The model under review builds one solid part; all positions refer to its coordinate system, in mm. Face numbers are marked on the shaded views. A direction names the side the tool comes from. Round coordinates to 2 decimals unless told otherwise and drop trailing zeros. Order: outer loops, then holes, each group sorted by start corner. A loop starts at its lowest first (then second) coordinate and runs counter-clockwise, first axis right, second up.
1) Clearance check with flat-ended pins moving along their axes: P1, Ø7.5, axis at x = -1, y = 19.5, coming from the +Z side; P2, Ø3, axis at y = 19.5, z = 0, coming from the -X side; P3, Ø14.5, axis at x = 29, y = 23.5, coming from the -Z side. State where each tip first meets the part, or that it passes through.
2) Consider section C-C (x = 5). Give the boundary of the cut face in (y, z) (3 decimals), then the cut area to 3 significant figures.
3) Mouldability with a two-part tool opening along Y and no side actions: class the marked faces 1, 2 and 3 as pulls with the +Y half, pulls with the -Y half, needs draft (parallel to the pull), parting line crosses it, or undercut.
4) Consider section B-B (y = 4). Give the boundary of the cut face in (x, z), then the cut area to 3 significant figures.
5) Consider section A-A (z = 17). Give the boundary of the cut face in (x, y).
6) To check wall thickness, follow L1, parallel to Y at x = 27, z = 17.25; L2, parallel to Y at x = 0, z = -14; L3, parallel to Y at x = 0, z = -12. State the ranges of each line that lie inside material, in increasing order.
7) Machinability: for the marked faces 4, 5, 6, 7 and 8, which of the approach directions +Z, -Z, +X, -X, +Y, -Y give a long, thin tool a straight path to every point of the face, cutting with its end or side? Answer none if there is none.
8) Consider section D-D (z = -4). Give the boundary of the cut face in (x, y).
from build123d import *

# Parameters (mm, degrees)
BOSS_EXTRUDE1_DEPTH   = 36
FILLET1_R             = 5
FILLET2_R             = 2
SKETCH2_R             = 3.5
CUT_EXTRUDE1_DEPTH    = 59.489315264
SKETCH3_R             = 10
CUT_EXTRUDE2_DEPTH    = 6
SKETCH4_R             = 8
BOSS_EXTRUDE2_DEPTH   = 11.09
M8_TAPPED_HOLE1_D     = 6.8
M8_TAPPED_HOLE1_DEPTH = 22.25
M8_TAPPED_HOLE1_TIP   = 2.042926105
FILLET3_R             = 2


with BuildPart() as part:
    # Sketch1 → Boss-Extrude1 (new body)
    with BuildSketch(Plane(origin=(0, 0, 0), x_dir=(1, 0, 0), z_dir=(0, 1, 0))):
        Polygon((-20, -13.744612069), (-20, 16.255387931), (20, 16.255387931), (20, -13.744612069), (35, -13.744612069), (35, -19.744612069), (18.390996312, -19.744612069), (10, -9.744612069), (-10, -9.744612069), (-18.390996312, -19.744612069), (-35, -19.744612069), (-35, -13.744612069), align=None)
        with BuildLine():
            Line((-10, 13.167446825), (10, 13.167446825))
            ThreePointArc((10, 13.167446825), (12, 11.167446825), (10, 9.167446825))
            Line((10, 9.167446825), (-10, 9.167446825))
            ThreePointArc((-10, 9.167446825), (-12, 11.167446825), (-10, 13.167446825))
        make_face(mode=Mode.SUBTRACT)
    extrude(amount=BOSS_EXTRUDE1_DEPTH)

    # Fillet1
    fillet1_edges = [part.edges().sort_by_distance(p)[0] for p in [
        (18.390996312, 18, 19.744612069),
        (10, 18, 9.744612069),
        (-10, 18, 9.744612069),
        (-18.390996312, 18, 19.744612069),
    ]]
    fillet(fillet1_edges, radius=FILLET1_R)

    # Fillet2
    fillet2_edges = [part.edges().sort_by_distance(p)[0] for p in [
        (20, 18, 13.744612069),
        (-20, 18, 13.744612069),
    ]]
    fillet(fillet2_edges, radius=FILLET2_R)

    # Sketch2 → Cut-Extrude1 (cut, through all)
    with BuildSketch(Plane(origin=(0, 0, 13.744612069), x_dir=(-1, 0, 0), z_dir=(0, 0, -1))):
        with Locations((-27, 18)):
            Circle(SKETCH2_R)
        with Locations((27, 18)):
            Circle(SKETCH2_R)
    extrude(amount=-CUT_EXTRUDE1_DEPTH, mode=Mode.SUBTRACT)

    # Sketch3 → Cut-Extrude2 (cut)
    with BuildSketch(Plane(origin=(0, 0, -16.255387931), x_dir=(-1, 0, 0), z_dir=(0, 0, -1))):
        with Locations((0, 18)):
            Circle(SKETCH3_R)
    extrude(amount=-CUT_EXTRUDE2_DEPTH, mode=Mode.SUBTRACT)

    # Sketch4 → Boss-Extrude2 (add)
    with BuildSketch(Plane(origin=(0, 0, -9.167446825), x_dir=(-1, 0, 0), z_dir=(0, 0, -1))):
        with Locations((0, 18)):
            Circle(SKETCH4_R)
    extrude(amount=BOSS_EXTRUDE2_DEPTH)

    # M8 Tapped Hole1
    with Locations(Plane(origin=(0, 0, -20.257446825), x_dir=(-1, 0, 0), z_dir=(0, 0, -1))):
        with Locations((0, 18)):
            Hole(M8_TAPPED_HOLE1_D / 2, depth=M8_TAPPED_HOLE1_DEPTH)
            with Locations((0, 0, -(M8_TAPPED_HOLE1_DEPTH + M8_TAPPED_HOLE1_TIP / 2))):  # 118° drill point
                Cone(0, M8_TAPPED_HOLE1_D / 2, M8_TAPPED_HOLE1_TIP, mode=Mode.SUBTRACT)

    # Fillet3
    fillet3_edges = [part.edges().sort_by_distance(p)[0] for p in [
        (-20, 18, -16.255387931),
        (20, 18, -16.255387931),
    ]]
    fillet(fillet3_edges, radius=FILLET3_R)


solid = part.part
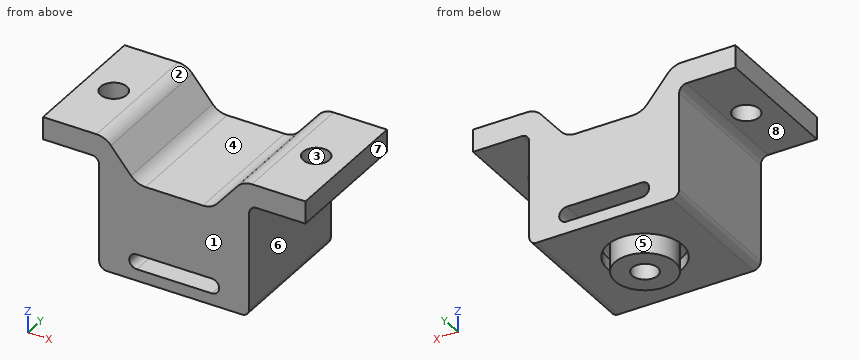
Answer below:
1. P1: stops at z = 9.74
1. P2: stops at x = -20
1. P3: stops at z = 13.73
2. outline: (0, -16.255) - (9.34, -16.255) - (9.34, -13.167) - (0, -13.167) - close; (0, -9.167) - (11.755, -9.167) - (11.755, -20.257) - (24.245, -20.257) - (24.245, -9.167) - (36, -9.167) - (36, 9.745) - (0, 9.745) - close; (26.66, -16.255) - (36, -16.255) - (36, -13.167) - (26.66, -13.167) - close
2. area: 877 mm2
3. face 1: pulls with the -Y half
3. face 2: needs draft
3. face 3: undercut
4. outline: (-35, 13.74) - (-22, 13.74) arc R2 cw to (-20, 11.74) - (-20, -14.26) arc R2 ccw to (-18, -16.26) - (18, -16.26) arc R2 ccw to (20, -14.26) - (20, 11.74) arc R2 cw to (22, 13.74) - (35, 13.74) - (35, 19.74) - (20.72, 19.74) arc R5 ccw to (16.89, 17.96) - (11.5, 11.53) arc R5 cw to (7.67, 9.74) - (-7.67, 9.74) arc R5 cw to (-11.5, 11.53) - (-16.89, 17.96) arc R5 ccw to (-20.72, 19.74) - (-35, 19.74) - close; hole (-10, -13.17) - (10, -13.17) arc R2 ccw to (10, -9.17) - (-10, -9.17) arc R2 ccw to start
4. area: 1,240 mm2
5. outline: (-35, 0) - (-16.09, 0) - (-16.09, 36) - (-35, 36) - close; (16.09, 0) - (35, 0) - (35, 36) - (16.09, 36) - close; hole circle Ø7 at (-27, 18); hole circle Ø7 at (27, 18)
6. L1: y = 0 to 14.5, 21.5 to 36
6. L2: y = 0 to 8, 10 to 14.6, 21.4 to 26, 28 to 36
6. L3: y = 10 to 14.6, 21.4 to 26
7. face 4: +Z, +Y, -Y
7. face 5: -Z
7. face 6: -Z, +X, +Y, -Y
7. face 7: +Z, -Z, +X, +Y, -Y
7. face 8: -Z, -X, +Y, -Y
8. outline: (-20, 0) - (20, 0) - (20, 36) - (-20, 36) - close; hole circle Ø6.8 at (0, 18)
